Read the model definition and answer for the solid it produces. Units are mm, in the model's axes. Give positions to 0.01 mm unless a question says otherwise; leave off trailing zeros. Put each result on its own line as item: value. Start each with the question number.
from build123d import *

# Parameters (mm, degrees)
SKETCH_1_R                = 200
EXTRUDE_1_DEPTH           = 10
SKETCH_2_R                = 125
CUT_EXTRUDE_1_DEPTH       = 284.548937575
HOLE_WIZARD_M12_1_D       = 10.2
PATTERN_CIRCULAR_1_COUNT  = 16
HOLE_WIZARD_1_D           = 11
HOLE_WIZARD_1_CBORE_D     = 18
HOLE_WIZARD_1_CBORE_DEPTH = 11
PATTERN_CIRCULAR_2_COUNT  = 4


with BuildPart() as part:
    # 草图1 → 凸台-拉伸1 (new, symmetric)
    with BuildSketch(Plane.XY):
        Circle(SKETCH_1_R)
    extrude(amount=EXTRUDE_1_DEPTH, both=True)

    # 草图2 → 切除-拉伸1 (cut, through all)
    with BuildSketch(Plane(origin=(0, 0, -10), x_dir=(-1, 0, 0), z_dir=(0, 0, -1))):
        Circle(SKETCH_2_R)
    extrude(amount=-CUT_EXTRUDE_1_DEPTH, mode=Mode.SUBTRACT)

    # M12 螺纹孔1 (through all)
    with Locations(Plane(origin=(0, 0, -10), x_dir=(-1, 0, 0), z_dir=(0, 0, -1))):
        with Locations((126.247255109, 121.188409419)):
            hole_wizard_m12_1 = Hole(HOLE_WIZARD_M12_1_D / 2)

    # 阵列(圆周)1: M12 螺纹孔1 ×16 about axis
    pattern_circular_1_axis = Axis((0, 0, 0), (0, 0, 1))
    for i in range(1, PATTERN_CIRCULAR_1_COUNT):
        add(hole_wizard_m12_1.rotate(pattern_circular_1_axis, i * 360 / PATTERN_CIRCULAR_1_COUNT), mode=Mode.SUBTRACT)

    # 打孔尺寸(%根据)内六角圆柱头螺钉的类型1 (through all)
    with Locations(Plane(origin=(0, 0, -10), x_dir=(-1, 0, 0), z_dir=(0, 0, -1))):
        with Locations((-164.950273467, 41.126722252)):
            hole_wizard_1 = CounterBoreHole(HOLE_WIZARD_1_D / 2, HOLE_WIZARD_1_CBORE_D / 2, HOLE_WIZARD_1_CBORE_DEPTH)

    # 阵列(圆周)2: 打孔尺寸(%根据)内六角圆柱头螺钉的类型1 ×4 about axis
    pattern_circular_2_axis = Axis((0, 0, 0), (0, 0, 1))
    for i in range(1, PATTERN_CIRCULAR_2_COUNT):
        add(hole_wizard_1.rotate(pattern_circular_2_axis, i * 360 / PATTERN_CIRCULAR_2_COUNT), mode=Mode.SUBTRACT)


solid = part.part
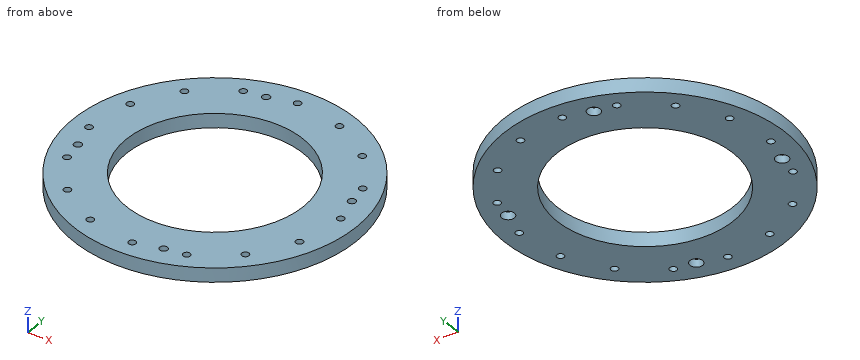
1) Each of these flat-tipped pins is pushed along its axis until it touches: pin 1 Ø16.5 at (x, y) = (-160.28, -70.26) entering from -Z; pin 2 Ø4 at (y, z) = (144, 5.5) entering from -X; pin 3 Ø12.5 at (x, y) = (-41.13, 164.95) entering from -Z; pin 4 Ø5 at (y, z) = (-153, -7) entering from +X. Where does it stop, or does it pass through?
2) A cutting plane is placed at A-A on z = -2. State how many separate pieces and enclosed holes the cut face has, and give its area (3 significant figures).
3) Straight lines are drawn through the part: line 1 (X direction, y = 48, z = -5); line 2 (Y direction, x = -38, z = -8.25); line 3 (Y direction, x = -160, z = 5.25). For each, find the intervals that lie inside material, in ascending order. Write a range as [from, to].
Results found:
1. pin 1: stops at z = -10
1. pin 2: stops at x = -140.84
1. pin 3: stops at z = 1
1. pin 4: stops at x = 131.72
2. separate pieces: 1
2. enclosed holes: 21
2. area: 74,300 mm²
3. line 1: x = [-194.15, -115.42], [115.42, 159.14], [170.76, 194.15]
3. line 2: y = [-196.36, -119.08], [119.08, 156.51], [173.39, 196.36]
3. line 3: y = [-120, -75.35], [-65.17, -43.52], [-38.73, 59.54], [67.76, 120]
